Check sheet for the modelled part. Datum: model origin and axes. Units: mm. A direction names the side the tool comes from. Round coordinates to 2 decimals unless told otherwise and drop trailing zeros. Write each loop counter-clockwise with the first axis right and the second up, starting at its lowest first coordinate (ties: lowest second). Pieces come first, ordered by that corner, then holes. Notation, with made-up numbers: (54.5, 4) -> (90.5, 4) arc R18 ccw to (90.5, 37) -> close; hole circle Ø11 at (7.5, 32.25). An arc over 180 degrees is marked (long way). Use one line per item in the form item = value. Start each with the question number.
```python
from build123d import *

# Parameters (mm, degrees)
SKETCH_1_W          = 600
SKETCH_1_H          = 150
EXTRUDE_1_DEPTH     = 1000
SHELL_1_T           = -2
SKETCH_3_W          = 596
SKETCH_3_H          = 148
CUT_EXTRUDE_1_DEPTH = 400
SKETCH_4_W          = 28
SKETCH_4_H          = 998
EXTRUDE_2_DEPTH     = 2
SKETCH_5_R          = 30
CUT_EXTRUDE_2_DEPTH = 2
SKETCH_6_W          = 540
SKETCH_6_H          = 120
CUT_EXTRUDE_3_DEPTH = 290
EXTRUDE_3_DEPTH     = 2
SKETCH_8_R          = 3
CUT_EXTRUDE_4_DEPTH = 1118
SKETCH_9_R          = 3
CUT_EXTRUDE_5_DEPTH = 10


with BuildPart() as part:
    # 草图1 → 凸台-拉伸1 (new body)
    with BuildSketch(Plane(origin=(0, 0, 0), x_dir=(1, 0, 0), z_dir=(0, 1, 0))):
        with Locations((300, 75)):
            Rectangle(SKETCH_1_W, SKETCH_1_H)
    extrude(amount=EXTRUDE_1_DEPTH)

    # 抽壳1
    shell_1_openings = [part.faces().sort_by_distance(p)[0] for p in [
        (300, 500, 0),
    ]]
    offset(amount=SHELL_1_T, openings=shell_1_openings, kind=Kind.INTERSECTION)

    # 草图3 → 切除-拉伸1 (cut)
    with BuildSketch(Plane.XZ):
        with Locations((300, -74)):
            Rectangle(SKETCH_3_W, SKETCH_3_H)
    extrude(amount=-CUT_EXTRUDE_1_DEPTH, mode=Mode.SUBTRACT)

    # 草图4 → 凸台-拉伸2 (add)
    with BuildSketch(Plane.XY):
        with Locations((16, 499)):
            Rectangle(SKETCH_4_W, SKETCH_4_H)
        with Locations((584, 499)):
            Rectangle(SKETCH_4_W, SKETCH_4_H)
    extrude(amount=-EXTRUDE_2_DEPTH)

    # 草图5 → 切除-拉伸2 (cut)
    with BuildSketch(Plane(origin=(0, 0, -150), x_dir=(-1, 0, 0), z_dir=(0, 0, -1))):
        with Locations((-150, 150)):
            Circle(SKETCH_5_R)
        with Locations((-150, 900)):
            Circle(SKETCH_5_R)
    extrude(amount=-CUT_EXTRUDE_2_DEPTH, mode=Mode.SUBTRACT)

    # 草图6 → 切除-拉伸3 (cut)
    with BuildSketch(Plane(origin=(0, 1000, 0), x_dir=(1, 0, 0), z_dir=(0, 1, 0))):
        with Locations((300, 60)):
            Rectangle(SKETCH_6_W, SKETCH_6_H)
    extrude(amount=-CUT_EXTRUDE_3_DEPTH, mode=Mode.SUBTRACT)

    # 草图7 → 凸台-拉伸3 (add)
    with BuildSketch(Plane.XZ):
        Polygon((0, 0), (0, -150), (600, -150), (600, 0), (570, 0), (570, -120), (30, -120), (30, 0), align=None)
    extrude(amount=-EXTRUDE_3_DEPTH)

    # 草图8 → 切除-拉伸4 (cut)
    with BuildSketch(Plane(origin=(0, 1000, 0), x_dir=(1, 0, 0), z_dir=(0, 1, 0))):
        with Locations(Location((15, 135, 0), (0, 0, 90))):
            Circle(SKETCH_8_R)
        with Locations(Location((343, 135, 0), (0, 0, 90))):
            Circle(SKETCH_8_R)
        with Locations(Location((585, 135, 0), (0, 0, 90))):
            Circle(SKETCH_8_R)
    extrude(amount=-CUT_EXTRUDE_4_DEPTH, mode=Mode.SUBTRACT)

    # 草图9 → 切除-拉伸5 (cut)
    with BuildSketch(Plane.XY):
        with Locations((15, 880)):
            Circle(SKETCH_9_R)
        with Locations((15, 30)):
            Circle(SKETCH_9_R)
        with Locations(Location((585, 880, 0), (0, 0, 180))):
            Circle(SKETCH_9_R)
        with Locations((15, 330)):
            Circle(SKETCH_9_R)
        with Locations(Location((585, 630, 0), (0, 0, 180))):
            Circle(SKETCH_9_R)
        with Locations((15, 630)):
            Circle(SKETCH_9_R)
        with Locations(Location((585, 330, 0), (0, 0, 180))):
            Circle(SKETCH_9_R)
        with Locations(Location((585, 30, 0), (0, 0, 180))):
            Circle(SKETCH_9_R)
    extrude(amount=-CUT_EXTRUDE_5_DEPTH, mode=Mode.SUBTRACT)


solid = part.part
```
1. Sectioned sample at D-D (x = 212.5). Enter the section's corners in (y, z), and give its area (3 significant figures).
2. Sectioned sample at C-C (y = 769.5). Enter the section's corners in (x, z).
3. Scan lines: probe 1 along X at (y, z) = (999, -135); probe 2 along Y at (x, z) = (150, -149); probe 3 along X at (y, z) = (880, -1.1). Record each from-to range of solid material in increasing order.
4. Sectioned sample at B-B (z = -60). Enter the section's corners in (x, y).
5. Depth check by flat-ended pin: pin 1 (1.5 mm diameter, centred on y = 859, z = -77, fed in from -X); pin 2 (5 mm diameter, centred on x = 585, y = 330, fed in from +Z); pin 3 (5 mm diameter, centred on x = 343, z = -135, fed in from -Y); pin 4 (1.6 mm diameter, centred on x = 330.5, y = 1, fed in from +Z). Enter the tip coordinate at first touch or a pass-through.
6. Sectioned sample at A-A (y = 900). Enter the section's corners in (x, z).
7. Mould release check, pull along X, two halves, no side actions. Record for faces 3 (the face through (600, 493, -74)), 4 (the face through (584, 507, -2)), 5 (the face through (299, 1000, -125)), 6 (the face through (153.905, 929.745, -149.014)): +X half, -X half, draft (parallel to the pull), parting line (faces both ways), or undercut.
8. Tool access check on faces 1 (the face through (296, 493, -150)), 2 (the face through (299, 2, -129)). Record the directions out of +Z, -Z, +X, -X, +Y, -Y that give a thin tool (end or side, any length) a straight path to the whole face; none if there is none.
Returned:
q1.outline = (0, -150) -> (1000, -150) -> (1000, -120) -> (998, -120) -> (998, -148) -> (2, -148) -> (2, -120) -> (0, -120) -> close
q1.area = 2,110 mm^2
q2.outline = (0, -150) -> (600, -150) -> (600, 0) -> (570, 0) -> (570, -2) -> (598, -2) -> (598, -148) -> (2, -148) -> (2, -2) -> (30, -2) -> (30, 0) -> (0, 0) -> close
q3.probe_1 = 0 to 12, 18 to 340, 346 to 582, 588 to 600
q3.probe_2 = 0 to 120, 180 to 870, 930 to 1000
q3.probe_3 = 0 to 12, 18 to 30, 570 to 582, 588 to 600
q4.outline = (0, 0) -> (30, 0) -> (30, 2) -> (2, 2) -> (2, 998) -> (30, 998) -> (30, 1000) -> (0, 1000) -> close; (570, 0) -> (600, 0) -> (600, 1000) -> (570, 1000) -> (570, 998) -> (598, 998) -> (598, 2) -> (570, 2) -> close
q5.pin_1 = 0
q5.pin_2 = -148
q5.pin_3 = through
q5.pin_4 = -120
q6.outline = (0, -150) -> (120, -150) -> (120, -148) -> (2, -148) -> (2, -2) -> (30, -2) -> (30, 0) -> (0, 0) -> close; (180, -150) -> (600, -150) -> (600, 0) -> (570, 0) -> (570, -2) -> (598, -2) -> (598, -148) -> (180, -148) -> close
q7.face_3 = +X half
q7.face_4 = undercut
q7.face_5 = draft
q7.face_6 = undercut
q8.face_1 = -Z, +X, -X, +Y, -Y
q8.face_2 = none
